from build123d import *

# Parameters (mm, degrees)
SKETCH1_R           = 12.5
BOSS_EXTRUDE1_DEPTH = 12
SKETCH2_OUTSIDE_W   = 35.546
SKETCH2_OUTSIDE_H   = 35.546
SKETCH2_OUTSIDE_R   = 4
CUT_EXTRUDE1_DEPTH  = 10
SKETCH9_OUTSIDE_W   = 35.546
SKETCH9_OUTSIDE_H   = 35.546
SKETCH9_OUTSIDE_W_2 = 15
SKETCH9_OUTSIDE_H_2 = 20
CUT_EXTRUDE2_DEPTH  = 30.807717122
M5_TAPPED_HOLE1_D   = 4.2
BOSS_EXTRUDE2_START = 2
SKETCH8_R           = 5
SKETCH8_R_2         = 4
BOSS_EXTRUDE2_DEPTH = 2
SKETCH6_W           = 3.5
SKETCH6_H           = 12.5
CHAMFER1_SIZE       = 0.5
CHAMFER2_SIZE       = 2
CHAMFER3_SIZE       = 1


with BuildPart() as part:
    # Sketch1 → Boss-Extrude1 (new, symmetric)
    with BuildSketch(Plane.XY):
        Circle(SKETCH1_R)
    extrude(amount=BOSS_EXTRUDE1_DEPTH, both=True)

    # Sketch2 outside → Cut-Extrude1 (cut)
    with BuildSketch(Plane.XY.offset(12)):
        Rectangle(SKETCH2_OUTSIDE_W, SKETCH2_OUTSIDE_H)
        Circle(SKETCH2_OUTSIDE_R, mode=Mode.SUBTRACT)
    extrude(amount=-CUT_EXTRUDE1_DEPTH, mode=Mode.SUBTRACT)

    # Sketch9 outside → Cut-Extrude2 (cut, through all)
    with BuildSketch(Plane(origin=(0, 0, -12), x_dir=(-1, 0, 0), z_dir=(0, 0, -1))):
        Rectangle(SKETCH9_OUTSIDE_W, SKETCH9_OUTSIDE_H)
        with Locations((0, 5)):
            Rectangle(SKETCH9_OUTSIDE_W_2, SKETCH9_OUTSIDE_H_2, mode=Mode.SUBTRACT)
    extrude(amount=-CUT_EXTRUDE2_DEPTH, mode=Mode.SUBTRACT)

    # M5 Tapped Hole1 (through all)
    with Locations(Plane(origin=(0, 0, -12), x_dir=(-1, 0, 0), z_dir=(0, 0, -1))):
        with Locations((0, 0)):
            Hole(M5_TAPPED_HOLE1_D / 2)

    # Sketch8 → Boss-Extrude2 (add)
    with BuildSketch(Plane.XY.offset(2).offset(BOSS_EXTRUDE2_START)):
        with Locations(Location((0, 0, 0), (0, 0, 270))):
            Circle(SKETCH8_R)
        Circle(SKETCH8_R_2, mode=Mode.SUBTRACT)
    extrude(amount=-BOSS_EXTRUDE2_DEPTH)

    # Sketch6 → M8x1.0 Tapped Hole1 (revolve, cut)
    with BuildSketch(Plane(origin=(0, 0, -5), x_dir=(0, 0, -1), z_dir=(1, 0, 0))):
        with Locations((1.75, 6.25)):
            Rectangle(SKETCH6_W, SKETCH6_H)
    revolve(axis=Axis((0, -6.35, -5), (0, 1, 0)), mode=Mode.SUBTRACT)

    # Chamfer1
    chamfer1_edges = [part.edges().sort_by_distance(p)[0] for p in [
        (-4, 0, 12),
        (0, 5, 4),
    ]]
    chamfer(chamfer1_edges, length=CHAMFER1_SIZE)

    # Chamfer2
    chamfer2_edges = [part.edges().sort_by_distance(p)[0] for p in [
        (-7.5, -5, -5),
        (7.5, -5, -5),
    ]]
    chamfer(chamfer2_edges, length=CHAMFER2_SIZE)

    # Chamfer3
    chamfer3_edges = [part.edges().sort_by_distance(p)[0] for p in [
        (0, 12.5, -12),
        (0, 12.5, 2),
    ]]
    chamfer(chamfer3_edges, length=CHAMFER3_SIZE)


solid = part.part
Verification items for the finished model (mm, model axes). A direction names the side the tool comes from. Round coordinates to 2 decimals unless told otherwise and drop trailing zeros. Order: outer loops, then holes, each group sorted by start corner. A loop starts at its lowest first (then second) coordinate and runs counter-clockwise, first axis right, second up. Notation, with made-up numbers: (-6, 37.25) -> (25, 37.25) arc R25 cw to (25, 58.25) -> close; hole circle Ø10 at (28, 54.25). An arc over 180 degrees is marked (long way). Put each result on its own line as item: value.
1) Section check D-D (z = -7.5). Record the cut outline in (x, y).
Final values:
outline: (-7.5, -3) -> (-5.5, -5) -> (5.5, -5) -> (7.5, -3) -> (7.5, 10) arc R12.5 ccw to (2.45, 12.26) -> (2.45, 0) -> (2.1, 0) arc R2.1 cw to (-2.1, 0) -> (-2.45, 0) -> (-2.45, 12.26) arc R12.5 ccw to (-7.5, 10) -> close
2) Set-up check for faces 1 (the cylindrical face through (-0.867, -3.905, 7.802)), 2 (the cylindrical face through (-0.154, 6.338, -1.503)), 3 (the conical face through (0.1, 11.7, 1.8)): record each of +Z, -Z, +X, -X, +Y, -Y from which the full face is reachable in a straight line by a thin tool's end or side.
Final values:
face 1: +Z
face 2: +Y
face 3: +Z, +Y
3) Mould release check, pull along Z, two halves, no side actions. Record for faces 4 (the flat face through (-0.1, 5.2, 2)), 5 (the cylindrical face through (-4.88, 1.08, 2.76)), 6 (the flat face through (-3, 0, -5)), 7 (the flat face through (0, 3, -12)): +Z half, -Z half, draft (parallel to the pull), parting line (faces both ways), or undercut.
Final values:
face 4: +Z half
face 5: draft
face 6: undercut
face 7: -Z half
4) Section check A-A (z = -10). Record the cut outline in (x, y), then the cut area to 3 significant figures.
Final values:
outline: (-7.5, -3) -> (-5.5, -5) -> (5.5, -5) -> (7.5, -3) -> (7.5, 10) arc R12.5 ccw to (-7.5, 10) -> close; hole circle Ø4.2 at (0, 0)
area: 233 mm^2
5) Material ranges on line 1 (Z direction, x = -4.75, y = 2.5); line 2 (Z direction, x = 0, y = 2.5); line 3 (X direction, y = 9.25, z = -5), recorded low to high.
Final values:
line 1: z = -12 to 2
line 2: z = -12 to -8.5, -1.5 to 12
line 3: x = -7.5 to -3.5, 3.5 to 7.5
6) Section check C-C (x = 1.25). Give the number of separate pieces and of enclosed holes in the cut face, then the cut area to 3 significant figures.
Final values:
separate pieces: 3
enclosed holes: 0
area: 171 mm^2
7) Section check B-B (z = -5). Record the cut outline in (x, y), then the cut area to 3 significant figures.
Final values:
outline: (-7.5, -3) -> (-5.5, -5) -> (5.5, -5) -> (7.5, -3) -> (7.5, 10) arc R12.5 ccw to (3.5, 12) -> (3.5, 0) -> (2.1, 0) arc R2.1 cw to (-2.1, 0) -> (-3.5, 0) -> (-3.5, 12) arc R12.5 ccw to (-7.5, 10) -> close
area: 153 mm^2
8) Depth check by flat-ended pin: pin 1 (1.5 mm diameter, centred on x = -1, y = 0.5, fed in from +Z); pin 2 (0.7 mm diameter, centred on x = -2.5, z = -5.5, fed in from +Y); pin 3 (6 mm diameter, centred on x = 3, z = -4.5, fed in from +Y); pin 4 (3 mm diameter, centred on x = -2.5, y = 3.5, fed in from +Z). Enter the tip coordinate at first touch or a pass-through.
Final values:
pin 1: passes through
pin 2: stops at y = 0
pin 3: stops at y = 12.4
pin 4: stops at z = 12
